Check sheet for the modelled part. Datum: model origin and axes. Units: mm. Round coordinates to 2 decimals unless told otherwise and drop trailing zeros. Write each loop counter-clockwise with the first axis right and the second up, starting at its lowest first coordinate (ties: lowest second). Pieces come first, ordered by that corner, then holes. Notation, with made-up numbers: M -26,32 L 14,32 A16 ccw 14,53 Z; hole C 47.5,-3 d2. An arc over 180 degrees is marked long. Answer in a Markdown table with one row per item.
```python
from build123d import *

# Parameters (mm, degrees)
SKETCH1_R           = 7.5
SKETCH1_R_2         = 4.5
BOSS_EXTRUDE1_DEPTH = 7.5


with BuildPart() as part:
    # Sketch1 → Boss-Extrude1 (new, symmetric)
    with BuildSketch(Plane.XY):
        with BuildLine():
            Line((0.80298849, 11.973103586), (67.5, 7.5))
            ThreePointArc((67.5, 7.5), (75, 0), (67.5, -7.5))
            Line((67.5, -7.5), (0.80298849, -11.973103586))
            ThreePointArc((0.80298849, -11.973103586), (-12, 0), (0.80298849, 11.973103586))
        make_face()
        Circle(SKETCH1_R, mode=Mode.SUBTRACT)
        with Locations((67.5, 0)):
            Circle(SKETCH1_R_2, mode=Mode.SUBTRACT)
    extrude(amount=BOSS_EXTRUDE1_DEPTH, both=True)


solid = part.part
```
1. Section check B-B, the plane x = 0. Record the cut outline in (y, z), and give its area (3 significant figures).
Found:
| item | result |
|---|---|
| outline | M -12,-7.5 L -7.5,-7.5 L -7.5,7.5 L -12,7.5 Z; M 7.5,-7.5 L 12,-7.5 L 12,7.5 L 7.5,7.5 Z |
| area | 135 mm2 |
2. Section check A-A, the plane y = 0. Record the cut outline in (x, z), and give its area (3 significant figures).
Found:
| item | result |
|---|---|
| outline | M -12,-7.5 L -7.5,-7.5 L -7.5,7.5 L -12,7.5 Z; M 7.5,-7.5 L 63,-7.5 L 63,7.5 L 7.5,7.5 Z; M 72,-7.5 L 75,-7.5 L 75,7.5 L 72,7.5 Z |
| area | 945 mm2 |
3. Go/stop test with flat-tipped pins: pin 1 (4 mm diameter, centred on y = -5, z = -2, fed in from -X); pin 2 (8 mm diameter, centred on x = 67.5, y = 0, fed in from +Z); pin 3 (1 mm diameter, centred on y = -5.5, z = -2, fed in from -X); pin 4 (3 mm diameter, centred on x = -3, z = -5, fed in from -Y). Record where each tip stops, or that it passes through.
Found:
| item | result |
|---|---|
| pin 1 | stops at x = -11.62 |
| pin 2 | passes through |
| pin 3 | stops at x = -10.91 |
| pin 4 | stops at y = -11.91 |
4. Section check D-D, the plane x = 66.5. Record the cut outline in (y, z).
Found:
| item | result |
|---|---|
| outline | M -7.57,-7.5 L -4.39,-7.5 L -4.39,7.5 L -7.57,7.5 Z; M 4.39,-7.5 L 7.57,-7.5 L 7.57,7.5 L 4.39,7.5 Z |
5. Section check C-C, the plane z = -2. Record the cut outline in (x, y).
Found:
| item | result |
|---|---|
| outline | M 0.8,-11.97 L 67.5,-7.5 A7.5 ccw 67.5,7.5 L 0.8,11.97 A12 ccw long Z; hole C 0,0 d15; hole C 67.5,0 d9 |
6. Draft check along X on faces 1 (the face through (-7.493, 0.33, -0.105)), 2 (the face through (32, 0, 7.5)), 3 (the face through (33.68, 9.77, 0.11)). Enter one of: +X half, -X half, draft (parallel to the pull), parting line (faces both ways), or undercut.
Found:
| item | result |
|---|---|
| face 1 | undercut |
| face 2 | draft |
| face 3 | +X half |
7. Scan lines: L1, parallel to X at y = -0.5, z = -2.75; L2, parallel to Y at x = 67.5, z = 4.5; L3, parallel to Y at x = 0, z = 2.25. Record each from-to range of solid material in increasing order.
Found:
| item | result |
|---|---|
| L1 | x = -11.99 to -7.48, 7.48 to 63.03, 71.97 to 74.98 |
| L2 | y = -7.5 to -4.5, 4.5 to 7.5 |
| L3 | y = -12 to -7.5, 7.5 to 12 |
